Input: part model. Units: mm. Frame: model coordinates. A direction names the side the tool comes from. Round coordinates to 2 decimals unless told otherwise and drop trailing zeros. Write each loop counter-clockwise with the first axis right and the second up, starting at its lowest first coordinate (ties: lowest second). Pieces come first, ordered by that corner, then holes. Notation, with made-up numbers: (40, 20) -> (75, 20) arc R29 cw to (75, 56) -> close; hole circle Ø8 at (9, 57). An arc over 180 degrees is marked (long way). Write item = value, one per line.
```python
from build123d import *

# Parameters (mm, degrees)
SKETCH_1_W                      = 220
SKETCH_1_H                      = 135
EXTRUDE_1_DEPTH                 = 12
HOLE_WIZARD_1_D                 = 6.6
HOLE_WIZARD_1_CBORE_D           = 11
HOLE_WIZARD_1_CBORE_DEPTH       = 6.8
SKETCH_4_W                      = 81
SKETCH_4_H                      = 135
CUT_EXTRUDE_1_DEPTH             = 2
HOLE_WIZARD_2_D                 = 6.6
HOLE_WIZARD_2_CBORE_D           = 11
HOLE_WIZARD_2_CBORE_DEPTH       = 6.8
HOLE_WIZARD_3_D                 = 6.6
HOLE_WIZARD_3_CBORE_D           = 11
HOLE_WIZARD_3_CBORE_DEPTH       = 6.8
CUT_EXTRUDE_2_REACH             = 131.616
SKETCH_9_R                      = 35
CUT_EXTRUDE_2_DIRECTION_2_DEPTH = 130.615778361
HOLE_WIZARD_M5_1_D              = 4.2
HOLE_WIZARD_M5_1_DEPTH          = 12.4
HOLE_WIZARD_M5_1_TIP            = 1.2618073


with BuildPart() as part:
    # 草图1 → 凸台-拉伸1 (new body)
    with BuildSketch(Plane.XY):
        Rectangle(SKETCH_1_W, SKETCH_1_H)
    extrude(amount=EXTRUDE_1_DEPTH)

    # 打孔尺寸(%根据)内六角圆柱头螺钉的类型1 (through all)
    with Locations(Plane.XY.offset(12)):
        with Locations((-91.500000058, 37.5), (-26.500000058, 37.5), (-91.500000058, -37.5), (-26.500000058, -37.5)):
            CounterBoreHole(HOLE_WIZARD_1_D / 2, HOLE_WIZARD_1_CBORE_D / 2, HOLE_WIZARD_1_CBORE_DEPTH)

    # 草图4 → 切除-拉伸1 (cut)
    with BuildSketch(Plane(origin=(0, 0, 0), x_dir=(-1, 0, 0), z_dir=(0, 0, -1))):
        with Locations((59.000000058, 0)):
            Rectangle(SKETCH_4_W, SKETCH_4_H)
    extrude(amount=-CUT_EXTRUDE_1_DEPTH, mode=Mode.SUBTRACT)

    # 打孔尺寸(%根据)内六角圆柱头螺钉的类型2 (through all)
    with Locations(Plane(origin=(0, 0, 2), x_dir=(-1, 0, 0), z_dir=(0, 0, -1))):
        with Locations((75, -32.5), (75, 27.5)):
            CounterBoreHole(HOLE_WIZARD_2_D / 2, HOLE_WIZARD_2_CBORE_D / 2, HOLE_WIZARD_2_CBORE_DEPTH)

    # 打孔尺寸(%根据)内六角圆柱头螺钉的类型3 (through all)
    with Locations(Plane(origin=(0, 0, 0), x_dir=(-1, 0, 0), z_dir=(0, 0, -1))):
        with Locations((-75, -32.5), (-75, 27.5)):
            CounterBoreHole(HOLE_WIZARD_3_D / 2, HOLE_WIZARD_3_CBORE_D / 2, HOLE_WIZARD_3_CBORE_DEPTH)

    # 草图9 → 切除-拉伸2 (cut, up to next)
    with BuildSketch(Plane(origin=(0, 0, 0), x_dir=(-1, 0, 0), z_dir=(0, 0, -1)), mode=Mode.PRIVATE) as cut_extrude_2_sk1:
        with Locations(Location((-25, 0, 0), (0, 0, 180))):
            Circle(SKETCH_9_R)
    cut_extrude_2_tool1 = extrude(cut_extrude_2_sk1.sketch, amount=-CUT_EXTRUDE_2_REACH, mode=Mode.PRIVATE) & part.part
    add(cut_extrude_2_tool1.solids().sort_by_distance((25, 0, 0))[0], mode=Mode.SUBTRACT)

    # 草图9 → 切除-拉伸2 direction 2 (cut)
    with BuildSketch(Plane(origin=(0, 0, 0), x_dir=(-1, 0, 0), z_dir=(0, 0, -1))):
        with Locations(Location((-25, 0, 0), (0, 0, 180))):
            Circle(SKETCH_9_R)
    extrude(amount=CUT_EXTRUDE_2_DIRECTION_2_DEPTH, mode=Mode.SUBTRACT)

    # M5 螺纹孔1
    with Locations(Plane(origin=(0, 67.5, 0), x_dir=(1, 0, 0), z_dir=(0, 1, 0))):
        with Locations((90, -6), (30, -6), (-102, -6)):
            Hole(HOLE_WIZARD_M5_1_D / 2, depth=HOLE_WIZARD_M5_1_DEPTH)
            with Locations((0, 0, -(HOLE_WIZARD_M5_1_DEPTH + HOLE_WIZARD_M5_1_TIP / 2))):  # 118° drill point
                Cone(0, HOLE_WIZARD_M5_1_D / 2, HOLE_WIZARD_M5_1_TIP, mode=Mode.SUBTRACT)


solid = part.part
```
1) First-contact query: P1, Ø7.5, axis at x = -26.5, y = -37.5, coming from the +Z side; P2, Ø3.5, axis at x = 90, z = 6, coming from the +Y side; P3, Ø2.5, axis at x = 30, z = 6, coming from the +Y side. Flat tips, straight axial feed; report the tip coordinate or a pass-through.
Solutions:
P1 = 5.2
P2 = 54.89
P3 = 54.59
2) Line query: L1, parallel to Y at x = -91, z = 4; L2, parallel to X at y = 38.5, z = 3; L3, parallel to X at y = -30.5, z = 10. Output: solid intervals per line, ascending. Write a range as from..to.
Solutions:
L1 = -67.5..-40.76, -34.24..34.24, 40.76..67.5
L2 = -110..-94.64, -88.36..-29.64, -23.36..110
L3 = -110..-77.62, -72.38..7.83, 42.17..72.38, 77.62..110
3) Draft query along Z for faces 1 (the face through (-27.216, -32.047, 8.648)), 2 (the face through (31.666, 61.213, 7.278)), 3 (the face through (59, 16, 0)). Return one class per face: +Z half, -Z half, draft (parallel to the pull), parting line (faces both ways), or undercut.
Solutions:
face_1 = draft
face_2 = undercut
face_3 = -Z half
4) Cut plane B-B (y = 0). Return the cut outline in (x, z), and give its area (3 significant figures).
Solutions:
outline = (-110, 0) -> (-99.5, 0) -> (-99.5, 2) -> (-18.5, 2) -> (-18.5, 0) -> (-10, 0) -> (-10, 12) -> (-110, 12) -> close; (60, 0) -> (110, 0) -> (110, 12) -> (60, 12) -> close
area = 1,640 mm^2
5) Cut plane C-C (y = 37.5). Return the cut outline in (x, z).
Solutions:
outline = (-110, 0) -> (-99.5, 0) -> (-99.5, 2) -> (-94.8, 2) -> (-94.8, 5.2) -> (-97, 5.2) -> (-97, 12) -> (-110, 12) -> close; (-88.2, 2) -> (-29.8, 2) -> (-29.8, 5.2) -> (-32, 5.2) -> (-32, 12) -> (-86, 12) -> (-86, 5.2) -> (-88.2, 5.2) -> close; (-23.2, 2) -> (-18.5, 2) -> (-18.5, 0) -> (110, 0) -> (110, 12) -> (-21, 12) -> (-21, 5.2) -> (-23.2, 5.2) -> close
6) Access query for faces 4 (the face through (71, 28, 6.8)), 5 (the face through (-94.65, 38.49, 3.58)), 6 (the face through (-86.254, 39.152, 8.648)). Directions: +Z, -Z, +X, -X, +Y, -Y. A direction counts if a zero-diameter tool reaches every point of the face in a straight line with its end or side. Return the directions, or none.
Solutions:
face_4 = -Z
face_5 = +Z, -Z
face_6 = +Z
7) Cut plane D-D (x = 25). Return the cut outline in (y, z).
Solutions:
outline = (-67.5, 0) -> (-35, 0) -> (-35, 12) -> (-67.5, 12) -> close; (35, 0) -> (67.5, 0) -> (67.5, 12) -> (35, 12) -> close
8) Cut plane A-A (x = 75). Return the cut outline in (y, z).
Solutions:
outline = (-67.5, 0) -> (-38, 0) -> (-38, 6.8) -> (-35.8, 6.8) -> (-35.8, 12) -> (-67.5, 12) -> close; (-29.2, 6.8) -> (-27, 6.8) -> (-27, 0) -> (22, 0) -> (22, 6.8) -> (24.2, 6.8) -> (24.2, 12) -> (-29.2, 12) -> close; (30.8, 6.8) -> (33, 6.8) -> (33, 0) -> (67.5, 0) -> (67.5, 12) -> (30.8, 12) -> close
